Answer from the drawing. Dimensions are ordinates in mm from the lowest x, y and z of the part. Give positions to 0.01 mm unless a question says otherwise; leave off trailing zeros. Use a Markdown table: item, result.
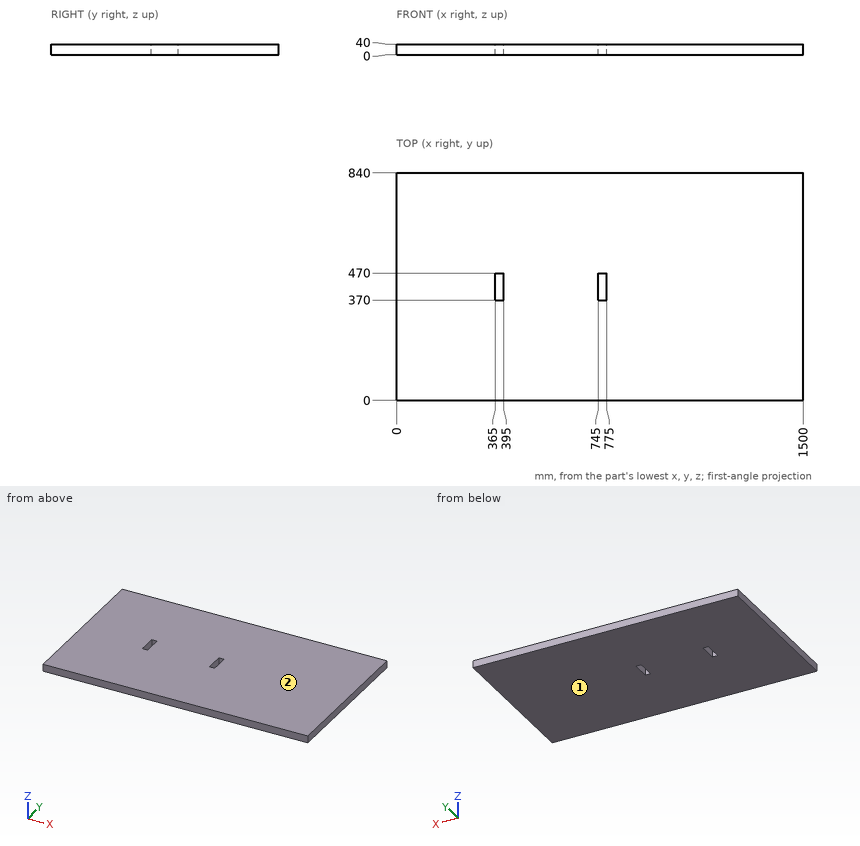
(1) Given P1, Ø2, axis at x = 1327, z = 22.5, coming from the -Y side, flat-ended and moving along its own axis, determine where the tip first touches the part or whether it passes through.
Entries:
| item | result |
|---|---|
| P1 | stops at y = 0 |
(2) Consider probe 1 along X at (y, z) = (422.5, 32.5); probe 2 along Y at (x, z) = (376, 36.5). Determine where each line is inside the solid, lowest interval first. Write a range as [from, to].
Entries:
| item | result |
|---|---|
| probe 1 | x = [0, 365], [395, 745], [775, 1500] |
| probe 2 | y = [0, 370], [470, 840] |
(3) The mould has two halves that part along Z. Classify the marked faces 1 and 2: released by +Z, released by -Z, zero draft, split by the parting line, or undercut.
Entries:
| item | result |
|---|---|
| face 1 | released by -Z |
| face 2 | released by +Z |
